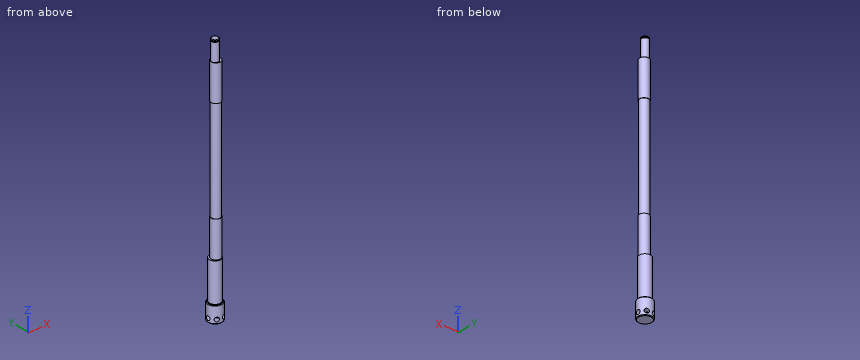
```python
from build123d import *

# Parameters (mm, degrees)
SKETCH1_R           = 6
BOSS_EXTRUDE1_DEPTH = 7
SKETCH2_R           = 4.75
BOSS_EXTRUDE2_DEPTH = 32
SKETCH3_R           = 4
BOSS_EXTRUDE3_DEPTH = 30
SKETCH4_R           = 3.75
BOSS_EXTRUDE4_DEPTH = 85
SKETCH5_R           = 4
BOSS_EXTRUDE5_DEPTH = 30
SKETCH6_R           = 3
BOSS_EXTRUDE6_DEPTH = 16.5
SKETCH8_W           = 1.531468115
SKETCH8_H           = 0.6
CHAMFER1_SIZE       = 0.5
SKETCH11_R          = 1.75
CUT_EXTRUDE1_DEPTH  = 11.5
CIRPATTERN1_COUNT   = 3
CIRPATTERN1_ANGLE   = 120
CHAMFER2_SIZE       = 0.5


with BuildPart() as part:
    # Sketch1 → Boss-Extrude1 (new, symmetric)
    with BuildSketch(Plane.XY):
        Circle(SKETCH1_R)
    extrude(amount=BOSS_EXTRUDE1_DEPTH, both=True)

    # Sketch2 → Boss-Extrude2 (add)
    with BuildSketch(Plane.XY.offset(7)):
        Circle(SKETCH2_R)
    extrude(amount=BOSS_EXTRUDE2_DEPTH)

    # Sketch3 → Boss-Extrude3 (add)
    with BuildSketch(Plane.XY.offset(39)):
        with Locations((0.75, 0)):
            Circle(SKETCH3_R)
    extrude(amount=BOSS_EXTRUDE3_DEPTH)

    # Sketch4 → Boss-Extrude4 (add)
    with BuildSketch(Plane.XY.offset(69)):
        with Locations((0.75, 0)):
            Circle(SKETCH4_R)
    extrude(amount=BOSS_EXTRUDE4_DEPTH)

    # Sketch5 → Boss-Extrude5 (add)
    with BuildSketch(Plane.XY.offset(154)):
        with Locations((0.75, 0)):
            Circle(SKETCH5_R)
    extrude(amount=BOSS_EXTRUDE5_DEPTH)

    # Sketch6 → Boss-Extrude6 (add)
    with BuildSketch(Plane.XY.offset(184)):
        Circle(SKETCH6_R)
    extrude(amount=BOSS_EXTRUDE6_DEPTH)

    # Sketch8 → Cut-Revolve1 (revolve, cut)
    with BuildSketch(Plane(origin=(0, 0, 0), x_dir=(1, 0, 0), z_dir=(0, 1, 0)), mode=Mode.PRIVATE) as cut_revolve1_sk:
        with Locations((3.565734058, -199.2)):
            Rectangle(SKETCH8_W, SKETCH8_H)
    revolve(cut_revolve1_sk.sketch.rotate(Axis((0, 0, 0), (0, 0, 1)), 180), axis=Axis((0, 0, 0), (0, 0, 1)), mode=Mode.SUBTRACT)

    # Chamfer1
    chamfer1_edges = [part.edges().sort_by_distance(p)[0] for p in [
        (-6, 0, -7),
        (-6, 0, 7),
    ]]
    chamfer(chamfer1_edges, length=CHAMFER1_SIZE)

    # Sketch11 → Cut-Extrude1 (cut, symmetric)
    with BuildSketch(Plane(origin=(0, 0, 0), x_dir=(0, 0, -1), z_dir=(1, 0, 0))):
        with Locations(Location((3.5, 0, 0), (0, 0, 180))):
            Circle(SKETCH11_R)
    cut_extrude1 = extrude(amount=CUT_EXTRUDE1_DEPTH, both=True, mode=Mode.SUBTRACT)

    # CirPattern1: Cut-Extrude1 ×3 about axis
    cirpattern1_axis = Axis((0, 0, 7), (0, 0, -1))
    for i in range(1, CIRPATTERN1_COUNT):
        add(cut_extrude1.rotate(cirpattern1_axis, i * CIRPATTERN1_ANGLE / (CIRPATTERN1_COUNT - 1)), mode=Mode.SUBTRACT)

    # Chamfer2
    chamfer2_edges = [part.edges().sort_by_distance(p)[0] for p in [
        (-3, 0, 200.5),
    ]]
    chamfer(chamfer2_edges, length=CHAMFER2_SIZE)


solid = part.part
```
Input: part model. Units: mm. Frame: model coordinates. Give positions to 0.01 mm unless a question says otherwise; leave off trailing zeros. Write each loop counter-clockwise with the first axis right and the second up, starting at its lowest first coordinate (ties: lowest second). Pieces come first, ordered by that corner, then holes. Notation, with made-up numbers: (26.5, 86) - (36.5, 86) arc R8 cw to (36.5, 91) - close; hole circle Ø10 at (89, -34). An arc over 180 degrees is marked (long way). Write item = value, one per line. Start each with the question number.
1. First-contact query: pin 1 Ø2 at (x, z) = (-3, 137) entering from -Y; pin 2 Ø6 at (y, z) = (3.5, 26) entering from -X; pin 3 Ø6 at (x, z) = (-1, 82) entering from +Y. Flat tips, straight axial feed; report the tip coordinate or a pass-through.
2. Ray query, L1, parallel to Y at x = 3.75, z = -3.5; L2, parallel to Z at x = 1, y = -1; L3, parallel to Y at x = 1, z = 75. Return the intervals inside material, ascending.
3. Section query B-B, the plane z = 11. Output: boundary loops of the cut face in (x, y).
4. Section query A-A, the plane z = 92. Output: boundary loops of the cut face in (x, y), then the cut area to 3 significant figures.
Check sheet entries:
q1.pin_1 = -2.55
q1.pin_2 = -4.72
q1.pin_3 = 3.75
q2.L1 = -3 to -1.75, 1.75 to 3
q2.L2 = -7 to -5.21, -1.79 to 200.5
q2.L3 = -3.74 to 3.74
q3.outline = circle Ø9.5 at (0, 0)
q4.outline = circle Ø7.5 at (0.75, 0)
q4.area = 44.2 mm2
